The model under review builds one solid part; all positions refer to its coordinate system, in mm. Face numbers are marked on the shaded views. A direction names the side the tool comes from. Round coordinates to 2 decimals unless told otherwise and drop trailing zeros. Loops run counter-clockwise (first coordinate to the right, second up) from the corner with the lowest first, then second, coordinate; pieces in that order, holes last. Notation, with made-up numbers: M 82,87.5 L 121,87.5 A24 ccw 121,113.5 Z; hole C 26,-0.75 d10. An arc over 180 degrees is marked long. Return JSON: item names as keys, results as strings. Group by question number.
Q1. Consider section D-D (x = 32). State the section outline as (y, z) points (3 decimals), and give its area (3 significant figures).
Q2. Draft analysis for pull direction X (two halves, no side actions). For the marked faces 1 and 2, state which applies: pulls with the +X half, pulls with the -X half, needs draft (parallel to the pull), parting line crosses it, or undercut.
Q3. Consider section C-C (y = -14). State the section outline as (x, z) points, and give its area (3 significant figures).
Q4. Clearance check with flat-ended pins moving along their axes: pin 1 Ø5 at (y, z) = (14, 13) entering from +X; pin 2 Ø14 at (x, z) = (32.5, 3) entering from +Y; pin 3 Ø12 at (x, z) = (82.5, -8) entering from +Y (3 decimals). State where each tip first meets the part, or that it passes through.
Q5. Consider section A-A (z = 0). State the section outline as (x, y) points (3 decimals).
Q6. Consider section B-B (x = 108.2). State the section outline as (y, z) points (3 decimals), and give its area (3 significant figures).
Q7. To check wall thickness, follow line 1 along Y through (x, z) = (0, -4); line 2 along X through (y, z) = (-14, -12.5); line 3 along Z through (x, y) = (108, -20). State the ranges of each line that lie inside material, in increasing order.
Q8. For the marked faces 3, 4, 5, 6 and 7, list the 3-axis set-ups (+Z, -Z, +X, -X, +Y, -Y) from which the entire face can be reached by the end or side of a thin tool; tool diameter is ignored.
from build123d import *

# Parameters (mm, degrees)
PIVOT_TUBE_SKETCH_R       = 26.5
PIVOT_TUBE_SKETCH_R_2     = 16.75
PIVOT_TUBE_53X_33_5_DEPTH = 28.25
ARM_PLATE_DEPTH           = 28.25
POST_SKETCH_R             = 38.1
POST_SKETCH_R_2           = 31.75
POST_BOSS_DEPTH           = 26.5
POST_TRIM_SKETCH_W        = 76.2
POST_TRIM_SKETCH_H        = 18.935
POST_TRIM_CUT_DEPTH       = 50
MOUNTING_PAD_SKETCH_R     = 31.75
MOUNTING_PAD_DEPTH        = 7.565
PAD_RECESS_SKETCH_R       = 31.75
PAD_RECESS_DEPTH          = 3.05
PAD_HOLE_SKETCH_R         = 10
PAD_HOLE_20_DEPTH         = 159.764275657
ARM_LINK_SKETCH_R         = 15
ARM_LINK_SKETCH_R_2       = 6.35
ARM_LINK_BOSS_DEPTH       = 49.815


with BuildPart() as part:
    # Pivot Tube Sketch → Pivot Tube Ø53xØ33.5 (new, symmetric)
    with BuildSketch(Plane.XY):
        Circle(PIVOT_TUBE_SKETCH_R)
        Circle(PIVOT_TUBE_SKETCH_R_2, mode=Mode.SUBTRACT)
    extrude(amount=PIVOT_TUBE_53X_33_5_DEPTH, both=True)

    # Arm Profile Sketch → Arm Plate (add, symmetric)
    with BuildSketch(Plane.XY):
        with BuildLine():
            Line((0, -26.5), (108.2, -26.5))
            Line((108.2, -26.5), (108.2, -18.935))
            Line((108.2, -18.935), (18.539573215, -18.935))
            ThreePointArc((18.539573215, -18.935), (10.011805531, -24.535968495), (0, -26.5))
        make_face()
    extrude(amount=ARM_PLATE_DEPTH, both=True)

    # Post Sketch → Post Boss (add)
    with BuildSketch(Plane(origin=(0, 0, 0), x_dir=(1, 0, 0), z_dir=(0, 1, 0))):
        with Locations(Location((108.2, 0, 0), (0, 0, 270))):
            Circle(POST_SKETCH_R)
        with Locations(Location((108.2, 0, 0), (0, 0, 270))):
            Circle(POST_SKETCH_R_2, mode=Mode.SUBTRACT)
    extrude(amount=-POST_BOSS_DEPTH)

    # Post Trim Sketch → Post Trim Cut (cut, symmetric)
    with BuildSketch(Plane.XY):
        with Locations((108.2, -9.4675)):
            Rectangle(POST_TRIM_SKETCH_W, POST_TRIM_SKETCH_H)
    extrude(amount=POST_TRIM_CUT_DEPTH, both=True, mode=Mode.SUBTRACT)

    # Mounting Pad Sketch → Mounting Pad (add)
    with BuildSketch(Plane(origin=(0, -18.935, 0), x_dir=(1, 0, 0), z_dir=(0, 1, 0))):
        with Locations((108.2, 0)):
            Circle(MOUNTING_PAD_SKETCH_R)
    extrude(amount=-MOUNTING_PAD_DEPTH)

    # Pad Recess Sketch → Pad Recess (cut)
    with BuildSketch(Plane(origin=(0, -18.935, 0), x_dir=(1, 0, 0), z_dir=(0, 1, 0))):
        with Locations(Location((108.2, 0, 0), (0, 0, 270))):
            Circle(PAD_RECESS_SKETCH_R)
    extrude(amount=-PAD_RECESS_DEPTH, mode=Mode.SUBTRACT)

    # Pad Hole Sketch → Pad Hole Ø20 (cut, through all)
    with BuildSketch(Plane(origin=(0, -21.985, 0), x_dir=(1, 0, 0), z_dir=(0, 1, 0))):
        with Locations(Location((108.2, 0, 0), (0, 0, 270))):
            Circle(PAD_HOLE_SKETCH_R)
    extrude(amount=-PAD_HOLE_20_DEPTH, mode=Mode.SUBTRACT)

    # Arm Link Sketch → Arm Link Boss (add)
    with BuildSketch(Plane(origin=(0, -18.935, 0), x_dir=(1, 0, 0), z_dir=(0, 1, 0))):
        with Locations(Location((32, 0, 0), (0, 0, 153.813423855))):
            Circle(ARM_LINK_SKETCH_R)
        with Locations(Location((32, 0, 0), (0, 0, 270))):
            Circle(ARM_LINK_SKETCH_R_2, mode=Mode.SUBTRACT)
    extrude(amount=ARM_LINK_BOSS_DEPTH)


solid = part.part
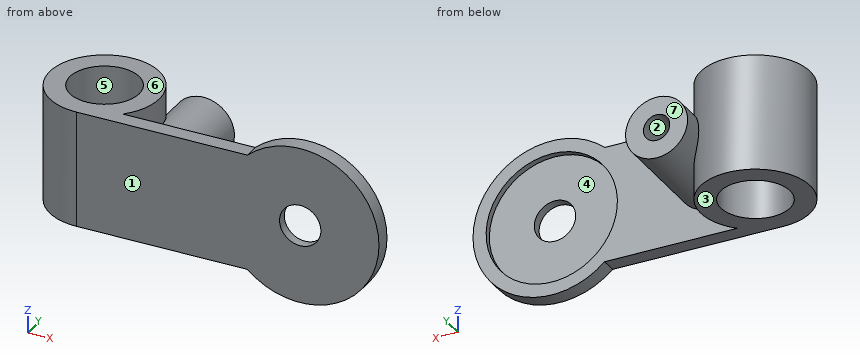
Values:
{
 "1": {"outline": "M -26.5,-28.25 L -18.935,-28.25 L -18.935,-15 L 30.88,-15 L 30.88,-6.35 L -18.935,-6.35 L -18.935,6.35 L 30.88,6.35 L 30.88,15 L -18.935,15 L -18.935,28.25 L -26.5,28.25 Z", "area": "1,290 mm2"},
 "2": {"face 1": "needs draft", "face 2": "undercut"},
 "3": {"outline": "M -22.5,-28.25 L -9.2,-28.25 L -9.2,28.25 L -22.5,28.25 Z; M 9.2,-28.25 L 22.5,-28.25 L 22.5,-11.61 A15 ccw long 22.5,11.61 L 22.5,28.25 L 9.2,28.25 Z; hole C 32,0 d12.7", "area": "1,990 mm2"},
 "4": {"pin 1": "stops at x = 42.71", "pin 2": "stops at y = 30.88", "pin 3": "stops at y = -18.935"},
 "5": {"outline": "M 0,-26.5 L 98.2,-26.5 L 98.2,-21.985 L 76.45,-21.985 L 76.45,-18.935 L 47,-18.935 L 47,30.88 L 38.35,30.88 L 38.35,-18.935 L 25.65,-18.935 L 25.65,-6.658 A26.5 ccw 25.65,6.658 L 25.65,30.88 L 17,30.88 L 17,20.329 A26.5 ccw long Z; M 118.2,-26.5 L 146.3,-26.5 L 146.3,-18.935 L 139.95,-18.935 L 139.95,-21.985 L 118.2,-21.985 Z; hole C 0,0 d33.5"},
 "6": {"outline": "M -26.5,-38.1 L -18.935,-38.1 L -18.935,-31.75 L -21.985,-31.75 L -21.985,-10 L -26.5,-10 Z; M -26.5,10 L -21.985,10 L -21.985,31.75 L -18.935,31.75 L -18.935,38.1 L -26.5,38.1 Z", "area": "292 mm2"},
 "7": {"line 1": "y = -26.5 to -16.75, 16.75 to 26.5", "line 2": "x = -22.5 to -9.2, 9.2 to 22.5, 23.71 to 40.29", "line 3": "z = -38.1 to -31.75, 31.75 to 38.1"},
 "8": {"face 3": "-Z, -X, +Y, -Y", "face 4": "+Y", "face 5": "+Z, -Z", "face 6": "+Z, -X, +Y, -Y", "face 7": "+Z, -Z, +X, -X, +Y"}
}
